The listing builds one solid part. Answer for the finished solid, in the listing's coordinates (mm). A direction names the side the tool comes from. Round coordinates to 2 decimals unless told otherwise and drop trailing zeros. Write each loop counter-clockwise with the first axis right and the second up, starting at its lowest first coordinate (ties: lowest second). Pieces come first, ordered by that corner, then holes. Notation, with made-up numbers: (-32.75, 78) - (-2.75, 78) arc R5 ccw to (-2.75, 84) - close; hole circle Ø3 at (-23.75, -6). An arc over 180 degrees is marked (long way). Answer in a Markdown table with one row per item.
from build123d import *

# Parameters (mm, degrees)
BASE_PLATE_DEPTH        = 10
SLOT_BOSS_DEPTH         = 22
SECONDARY_BOSS_DEPTH    = 10
SLOT_CUT_SKETCH_R       = 5
SLOT_THROUGH_CUT_DEPTH  = 34.5
COUNTERBORE_SKETCH_R    = 6.5
COUNTERBORES_6X_DEPTH   = 3
MOUNTING_HOLE_SKETCH_R  = 3
MOUNTING_HOLES_6X_DEPTH = 88


with BuildPart() as part:
    # Base Plate Sketch → Base Plate (new body)
    with BuildSketch(Plane(origin=(0, 0, 0), x_dir=(1, 0, 0), z_dir=(0, 1, 0))):
        with BuildLine():
            Line((40, 22), (40, -22))
            ThreePointArc((40, -22), (0, -62), (-40, -22))
            Line((-40, -22), (-40, 22))
            ThreePointArc((-40, 22), (0, 62), (40, 22))
        make_face()
    extrude(amount=BASE_PLATE_DEPTH)

    # Slot Boss Sketch → Slot Boss (add)
    with BuildSketch(Plane(origin=(0, 10, 0), x_dir=(1, 0, 0), z_dir=(0, 1, 0))):
        with BuildLine():
            Line((16, 22), (16, -22))
            ThreePointArc((16, -22), (0, -38), (-16, -22))
            Line((-16, -22), (-16, 22))
            ThreePointArc((-16, 22), (0, 38), (16, 22))
        make_face()
        with BuildLine():
            Line((10, 22), (10, -22))
            ThreePointArc((10, -22), (0, -32), (-10, -22))
            Line((-10, -22), (-10, 22))
            ThreePointArc((-10, 22), (0, 32), (10, 22))
        make_face(mode=Mode.SUBTRACT)
    extrude(amount=SLOT_BOSS_DEPTH)

    # Secondary Boss Sketch → Secondary Boss (add)
    with BuildSketch(Plane(origin=(0, 10, 0), x_dir=(1, 0, 0), z_dir=(0, 1, 0))):
        with BuildLine():
            Line((-10, 22), (-10, -22))
            ThreePointArc((-10, -22), (0, -32), (10, -22))
            Line((10, -22), (10, 22))
            ThreePointArc((10, 22), (0, 32), (-10, 22))
        make_face()
    extrude(amount=SECONDARY_BOSS_DEPTH)

    # Slot Cut Sketch → Slot Through Cut (cut, symmetric)
    with BuildSketch(Plane(origin=(0, 10, 0), x_dir=(1, 0, 0), z_dir=(0, 1, 0))):
        with Locations(Location((0, 22, 0), (0, 0, 270))):
            Circle(SLOT_CUT_SKETCH_R)
        with Locations(Location((0, -22, 0), (0, 0, 270))):
            Circle(SLOT_CUT_SKETCH_R)
    extrude(amount=SLOT_THROUGH_CUT_DEPTH, both=True, mode=Mode.SUBTRACT)

    # Counterbore Sketch → Counterbores 6x (cut)
    with BuildSketch(Plane(origin=(0, 10, 0), x_dir=(1, 0, 0), z_dir=(0, 1, 0))):
        with Locations(Location((0, -48, 0), (0, 0, 270))):
            Circle(COUNTERBORE_SKETCH_R)
        with Locations(Location((0, 48, 0), (0, 0, 270))):
            Circle(COUNTERBORE_SKETCH_R)
        with Locations(Location((26, -22, 0), (0, 0, 270))):
            Circle(COUNTERBORE_SKETCH_R)
        with Locations(Location((-26, -22, 0), (0, 0, 270))):
            Circle(COUNTERBORE_SKETCH_R)
        with Locations(Location((26, 22, 0), (0, 0, 90))):
            Circle(COUNTERBORE_SKETCH_R)
        with Locations(Location((-26, 22, 0), (0, 0, 90))):
            Circle(COUNTERBORE_SKETCH_R)
    extrude(amount=-COUNTERBORES_6X_DEPTH, mode=Mode.SUBTRACT)

    # Mounting Hole Sketch → Mounting Holes 6x (cut)
    with BuildSketch(Plane(origin=(0, 10, 0), x_dir=(1, 0, 0), z_dir=(0, 1, 0))):
        with Locations(Location((0, -48, 0), (0, 0, 270))):
            Circle(MOUNTING_HOLE_SKETCH_R)
        with Locations(Location((26, -22, 0), (0, 0, 270))):
            Circle(MOUNTING_HOLE_SKETCH_R)
        with Locations(Location((26, 22, 0), (0, 0, 270))):
            Circle(MOUNTING_HOLE_SKETCH_R)
        with Locations(Location((0, 48, 0), (0, 0, 270))):
            Circle(MOUNTING_HOLE_SKETCH_R)
        with Locations(Location((-26, 22, 0), (0, 0, 270))):
            Circle(MOUNTING_HOLE_SKETCH_R)
        with Locations(Location((-26, -22, 0), (0, 0, 270))):
            Circle(MOUNTING_HOLE_SKETCH_R)
    extrude(amount=-MOUNTING_HOLES_6X_DEPTH, mode=Mode.SUBTRACT)


solid = part.part
(1) Section A-A (y = 23) is taken. Give the vertices of the cut face in (x, z).
Checked values:
| item | result |
|---|---|
| outline | (-16, -22) arc R16 ccw to (16, -22) - (16, 22) arc R16 ccw to (-16, 22) - close; hole (-10, -22) arc R10 ccw to (10, -22) - (10, 22) arc R10 ccw to (-10, 22) - close |
(2) Section C-C (x = -26) is taken. Give the vertices of the cut face in (y, z), and give its area (3 significant figures).
Checked values:
| item | result |
|---|---|
| outline | (0, -52.4) - (10, -52.4) - (10, -28.5) - (7, -28.5) - (7, -25) - (0, -25) - close; (0, -19) - (7, -19) - (7, -15.5) - (10, -15.5) - (10, 15.5) - (7, 15.5) - (7, 19) - (0, 19) - close; (0, 25) - (7, 25) - (7, 28.5) - (10, 28.5) - (10, 52.4) - (0, 52.4) - close |
| area | 886 mm2 |
(3) Flat-ended cylindrical pins translate along their axes: pin 1 (13 mm diameter, centred on y = 24.5, z = -5, fed in from +X); pin 2 (3 mm diameter, centred on y = 12.5, z = -44, fed in from -X); pin 3 (15 mm diameter, centred on x = -26, z = 22, fed in from +Y); pin 4 (2 mm diameter, centred on y = 26, z = 33, fed in from +X). Find the tip coordinate at first contact, or state that the pin passes through.
Checked values:
| item | result |
|---|---|
| pin 1 | stops at x = 16 |
| pin 2 | passes through |
| pin 3 | stops at y = 10 |
| pin 4 | stops at x = 12.49 |
(4) Find the intervals of material crossed by line 1 (X direction, y = 1.75, z = -22); line 2 (X direction, y = 8, z = 22); line 3 (Z direction, x = 4, y = 4.5), in increasing order.
Checked values:
| item | result |
|---|---|
| line 1 | x = -40 to -29, -23 to -5, 5 to 23, 29 to 40 |
| line 2 | x = -40 to -32.5, -19.5 to -5, 5 to 19.5, 32.5 to 40 |
| line 3 | z = -61.8 to -25, -19 to 19, 25 to 61.8 |
(5) For a pull along X with two mould halves and no side action, classify faces 1 (the flat face through (-17, 10, -1)), 2 (the cylindrical face through (-26.286, 8.521, -15.506)), 3 (the cylindrical face through (0, 21, 38)) as pulls with the +X half, pulls with the -X half, needs draft (parallel to the pull), parting line crosses it, or undercut.
Checked values:
| item | result |
|---|---|
| face 1 | needs draft |
| face 2 | undercut |
| face 3 | parting line crosses it |
(6) Section B-B (z = 48) is taken. Give the vertices of the cut face in (x, y).
Checked values:
| item | result |
|---|---|
| outline | (-30.4, 0) - (-3, 0) - (-3, 7) - (-6.5, 7) - (-6.5, 10) - (-30.4, 10) - close; (3, 0) - (30.4, 0) - (30.4, 10) - (6.5, 10) - (6.5, 7) - (3, 7) - close |
(7) Section D-D (y = 2) is taken. State how many separate pieces and enclosed holes the cut face has, and give its area (3 significant figures).
Checked values:
| item | result |
|---|---|
| separate pieces | 1 |
| enclosed holes | 8 |
| area | 8,220 mm2 |
(8) For faces 4 (the cylindrical face through (0, 10, 17)), 5 (the cylindrical face through (-25.714, 8.521, 15.506)), determine the directions among +Z, -Z, +X, -X, +Y, -Y from which every point of the face is accessible in a straight line to the end or side of a thin tool.
Checked values:
| item | result |
|---|---|
| face 4 | +Y, -Y |
| face 5 | +Y |
